Part model, mm, in its own coordinate system. A direction names the side the tool comes from. Round coordinates to 2 decimals unless told otherwise and drop trailing zeros. Loops run counter-clockwise (first coordinate to the right, second up) from the corner with the lowest first, then second, coordinate; pieces in that order, holes last. Notation, with made-up numbers: M 83,16.25 L 125,16.25 A21 cw 125,42.25 Z; hole C 3.25,85.25 d5. An arc over 180 degrees is marked long. Put each result on its own line as item: value. Start each with the question number.
1) Slice it at B-B on z = 351.5. Give the cut face in (x, y).
2) Pull direction Y, two halves, no side cores. Call faces 3 (the flat face through (-34.54, -228.12, 419.05)), 4 (the flat face through (-77, -119, 0)), 5 (the flat face through (-42, 0, 419)): +Y half, -Y half, draft (parallel to the pull), parting line (faces both ways), or undercut.
3) Probe line 1 along X through (y, z) = (-44, 556.5); line 2 along Y through (x, z) = (-39, 509.5); line 3 along Y through (x, z) = (-52, 504). List the from-to ranges inside material, lowest first.
4) Drop a flat-ended pin along its axis: pin 1 Ø12 at (y, z) = (-212.5, 444) entering from +X. Give the stop position or say it passes through.
5) Slice it at C-C on y = -77. Give the cut face in (x, z).
6) Slice it at A-A on x = -24. Give the cut face in (y, z).
7) Which spindle directions (+Z, -Z, +X, -X, +Y, -Y) get a long thin tool onto all of the face, cutting with end or side? Do faces 1 (the flat face through (-85, -118, 419)), 2 (the flat face through (-35.363, -11.997, 419.05)). Say none if no direction does.
```python
from build123d import *

# Parameters (mm, degrees)
EXTRUDE_1_DEPTH = 850


with BuildPart() as part:
    # 草图1 → 凸台-拉伸1 (new body)
    with BuildSketch(Plane.XY):
        with BuildLine():
            Line((0, 0), (-85, 0))
            Line((-85, 0), (-85, -240))
            Line((-85, -240), (0, -240))
            Line((0, -240), (0, -238.623349271))
            ThreePointArc((0, -238.623349271), (-1.594387729, -234.358965582), (-5.595374844, -232.186606824))
            Line((-5.595374844, -232.186606824), (-64.309250312, -223.934909757))
            ThreePointArc((-64.309250312, -223.934909757), (-72.311224543, -219.59019224), (-75.5, -211.061424863))
            Line((-75.5, -211.061424863), (-75.5, -28.938575137))
            ThreePointArc((-75.5, -28.938575137), (-72.311224543, -20.40980776), (-64.309250312, -16.065090243))
            Line((-64.309250312, -16.065090243), (-5.595374844, -7.813393176))
            ThreePointArc((-5.595374844, -7.813393176), (-1.594387729, -5.641034418), (0, -1.376650729))
            Line((0, -1.376650729), (0, 0))
        make_face()
    extrude(amount=EXTRUDE_1_DEPTH)


solid = part.part
```
Recorded:
1. outline: M -85,-240 L 0,-240 L 0,-238.62 A6.5 ccw -5.6,-232.19 L -64.31,-223.93 A13 cw -75.5,-211.06 L -75.5,-28.94 A13 cw -64.31,-16.07 L -5.6,-7.81 A6.5 ccw 0,-1.38 L 0,0 L -85,0 Z
2. face 3: undercut
2. face 4: draft
2. face 5: +Y half
3. line 1: x = -85 to -75.5
3. line 2: y = -240 to -227.49, -12.51 to 0
3. line 3: y = -240 to -225.66, -14.34 to 0
4. pin 1: stops at x = -73.16
5. outline: M -85,0 L -75.5,0 L -75.5,850 L -85,850 Z
6. outline: M -240,0 L -229.6,0 L -229.6,850 L -240,850 Z; M -10.4,0 L 0,0 L 0,850 L -10.4,850 Z
7. face 1: +Z, -Z, -X, +Y, -Y
7. face 2: +Z, -Z, +X
